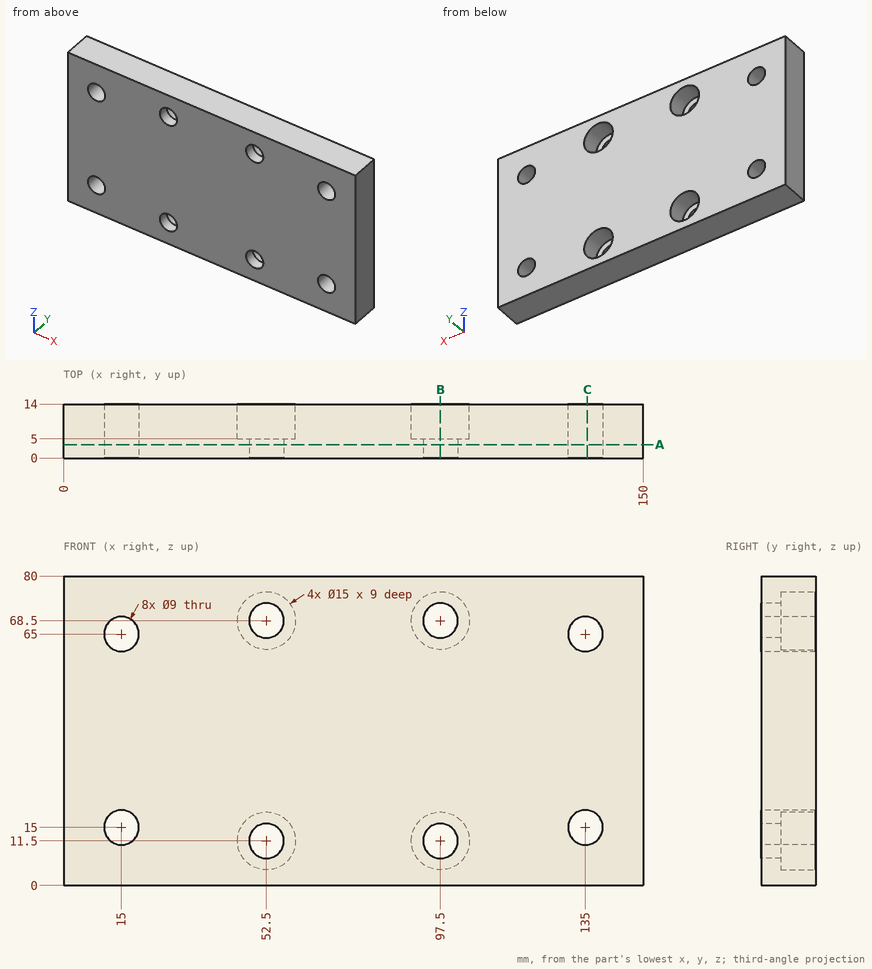
Could you check a few things on this drawing? It's one solid part, dimensions in mm from its lowest x, y, z. Round coordinates to 2 decimals unless told otherwise and drop trailing zeros. Order: outer loops, then holes, each group sorted by start corner. A loop starts at its lowest first (then second) coordinate and runs counter-clockwise, first axis right, second up. Notation, with made-up numbers: M -19,-17 L 17,-17 A20 cw 17,-1 Z; hole C 53,-34.75 d4. An arc over 180 degrees is marked long. One line per question, with ' | ' between items. Start each with the question number.
(1) Suppose I cut it at A-A on y = 3.5. Count the separate pieces of the cut face and the enclosed holes in it, then the cut area to 3 significant figures.
(2) Suppose I cut it at C-C on x = 135.5. List the corners of the cut face in (y, z) for me, then the cut area to 3 significant figures.
(3) Suppose I cut it at B-B on x = 97.5. List the corners of the cut face in (y, z) for me, then the cut area to 3 significant figures.
(4) Please list where these lines run through material, in increasing order: line 1 along Z through (x, y) = (52.5, 3.85); line 2 along Z through (x, y) = (135, 6.25); line 3 along X through (y, z) = (4.5, 67.5).
(5) For P1, Ø11.5, axis at x = 97.5, z = 11.5, coming from the +Y side, with a flat end and sliding along its axis, tell me the tip position at first contact or that it passes through.
Geometry results:
1) separate pieces: 1 | enclosed holes: 8 | area: 11,500 mm²
2) outline: M 0,0 L 14,0 L 14,10.53 L 0,10.53 Z; M 0,19.47 L 14,19.47 L 14,60.53 L 0,60.53 Z; M 0,69.47 L 14,69.47 L 14,80 L 0,80 Z | area: 870 mm²
3) outline: M 0,0 L 14,0 L 14,4 L 5,4 L 5,7 L 0,7 Z; M 0,16 L 5,16 L 5,19 L 14,19 L 14,61 L 5,61 L 5,64 L 0,64 Z; M 0,73 L 5,73 L 5,76 L 14,76 L 14,80 L 0,80 Z | area: 760 mm²
4) line 1: 0 to 7, 16 to 64, 73 to 80 | line 2: 0 to 10.5, 19.5 to 60.5, 69.5 to 80 | line 3: 0 to 11.26, 18.74 to 48.11, 56.89 to 93.11, 101.89 to 131.26, 138.74 to 150
5) P1: y = 5
